```python
from build123d import *

# Parameters (mm, degrees)
SKETCH_1_W         = 6
SKETCH_1_H         = 6
EXTRUDE_1_DEPTH    = 20
HOLE_WIZARD_M3_1_D = 2.5
HOLE_WIZARD_M3_2_D = 2.5
FILLET_1_R         = 0.5


with BuildPart() as part:
    # 草图1 → 凸台-拉伸1 (new, symmetric)
    with BuildSketch(Plane.XY):
        Rectangle(SKETCH_1_W, SKETCH_1_H)
    extrude(amount=EXTRUDE_1_DEPTH, both=True)

    # M3 螺纹孔1 (through all)
    with Locations(Plane(origin=(0, 3, 0), x_dir=(1, 0, 0), z_dir=(0, 1, 0))):
        with Locations((0, 15), (0, -5)):
            Hole(HOLE_WIZARD_M3_1_D / 2)

    # M3 螺纹孔2 (through all)
    with Locations(Plane(origin=(3, 0, 0), x_dir=(0, 0, -1), z_dir=(1, 0, 0))):
        with Locations((-15, 0), (5, 0)):
            Hole(HOLE_WIZARD_M3_2_D / 2)

    # 圆角1
    fillet_1_edges = [part.edges().sort_by_distance(p)[0] for p in [
        (3, -3, 0),
        (-3, -3, 0),
        (-3, 3, 0),
        (3, 3, 0),
    ]]
    fillet(fillet_1_edges, radius=FILLET_1_R)


solid = part.part
```
Model file for the job. Use its own axes, mm. Coordinates: 2 decimals unless noted, no trailing zeros. Order: outer loops, then holes, each group sorted by start corner. A loop starts at its lowest first (then second) coordinate and runs counter-clockwise, first axis right, second up. Notation, with made-up numbers: M 54.5,25.5 L 75.5,25.5 A25 ccw 75.5,53.5 Z; hole C 80.25,54 d6. An arc over 180 degrees is marked long. Answer as CSV lines item,"result".
(1) Band-saw the part on A-A, the plane y = 0. List the corners of the cut face in (x, z), then the cut area to 3 significant figures.
Geometry says:
outline,"M -3,-20 L 3,-20 L 3,-6.25 L -3,-6.25 Z; M -3,-3.75 L 3,-3.75 L 3,13.75 L -3,13.75 Z; M -3,16.25 L 3,16.25 L 3,20 L -3,20 Z; hole C 0,-15 d2.5; hole C 0,5 d2.5"
area,"200 mm2"
(2) Band-saw the part on B-B, the plane z = 5. List the corners of the cut face in (x, y).
Geometry says:
outline,"M -3,-2.5 A0.5 ccw -2.5,-3 L -1.25,-3 L -1.25,3 L -2.5,3 A0.5 ccw -3,2.5 Z; M 1.25,-3 L 2.5,-3 A0.5 ccw 3,-2.5 L 3,2.5 A0.5 ccw 2.5,3 L 1.25,3 Z"
(3) Band-saw the part on C-C, the plane x = -0.35. List the corners of the cut face in (y, z), then the cut area to 3 significant figures.
Geometry says:
outline,"M -3,-20 L 3,-20 L 3,-16.2 L -3,-16.2 Z; M -3,-13.8 L 3,-13.8 L 3,3.8 L -3,3.8 Z; M -3,6.2 L 3,6.2 L 3,20 L -3,20 Z; hole C 0,-5 d2.5; hole C 0,15 d2.5"
area,"201 mm2"
(4) Flat gauge pin, fed straight in: pin 1 (3 mm diameter, centred on x = 0, z = 5, fed in from -Y). Where does the tip first touch, or does it go through?
Geometry says:
pin 1,"stops at y = -3"
(5) Wall check: line 1 along Y through (x, z) = (-0.4, -5); line 2 along Z through (x, y) = (0.4, 0.8); line 3 along Z through (x, y) = (0.15, -2.6). Give the ranges that are in metal, low to high.
Geometry says:
line 1,"y = -3 to -1.25, 1.25 to 3"
line 2,"z = -20 to -16.18, -13.82 to -5.96, -4.04 to 3.82, 6.18 to 14.04, 15.96 to 20"
line 3,"z = -20 to -16.24, -13.76 to 3.76, 6.24 to 20"
(6) Band-saw the part on D-D, the plane y = 2. List the corners of the cut face in (x, z), then the cut area to 3 significant figures.
Geometry says:
outline,"M -3,-20 L 3,-20 L 3,20 L -3,20 Z; hole C 0,-15 d2.5; hole C 0,5 d2.5"
area,"230 mm2"
(7) Pull direction Z, two halves, no side cores. Call faces 1 (the cylindrical face through (0.27, -0.04, 6.22)), 2 (the flat face through (0, 0, -20)), 3 (the flat face through (0, 3, 0)): +Z half, -Z half, draft (parallel to the pull), parting line (faces both ways), or undercut.
Geometry says:
face 1,"undercut"
face 2,"-Z half"
face 3,"draft"
